from build123d import *

# Parameters (mm, degrees)
SKETCH_1_W                   = 64
SKETCH_1_H                   = 45
EXTRUDE_1_DEPTH              = 11.5
HOLE_WIZARD_M4_1_D           = 4.5
HOLE_WIZARD_M4_1_CBORE_D     = 8
HOLE_WIZARD_M4_1_CBORE_DEPTH = 4.4
FILLET_1_R                   = 3


with BuildPart() as part:
    # 草图1 → 凸台-拉伸1 (new, symmetric)
    with BuildSketch(Plane(origin=(0, 0, 0), x_dir=(1, 0, 0), z_dir=(0, 1, 0))):
        Rectangle(SKETCH_1_W, SKETCH_1_H)
    extrude(amount=EXTRUDE_1_DEPTH, both=True)

    # M4 六角凹头螺钉的柱形沉头孔1 (through all)
    with Locations(Plane(origin=(0, 11.5, 0), x_dir=(1, 0, 0), z_dir=(0, 1, 0))):
        with Locations((-23.5, 0), (23.5, 0)):
            CounterBoreHole(HOLE_WIZARD_M4_1_D / 2, HOLE_WIZARD_M4_1_CBORE_D / 2, HOLE_WIZARD_M4_1_CBORE_DEPTH)

    # 圆角1
    fillet_1_edges = [part.edges().sort_by_distance(p)[0] for p in [
        (32, 0, 22.5),
        (-32, 0, 22.5),
        (-32, 0, -22.5),
        (32, 0, -22.5),
    ]]
    fillet(fillet_1_edges, radius=FILLET_1_R)


solid = part.part
Could you check a few things on this model? Use its own coordinates, in mm. A direction names the side the tool comes from. Coordinates: 2 decimals unless noted, no trailing zeros. Loops run counter-clockwise (first coordinate to the right, second up) from the corner with the lowest first, then second, coordinate; pieces in that order, holes last.
1. For P1, Ø7, axis at x = 23.5, z = 0, coming from the +Y side, with a flat end and sliding along its axis, tell me the tip position at first contact or that it passes through.
2. Imagine slicing it at C-C (z = 0). Please give me the cut outline in (x, y), and give its area (3 significant figures).
3. Imagine slicing it at B-B (y = 8). Please give me the cut outline in (x, z).
4. For faces 4 (the face through (-22, 7.1, 2)), 5 (the face through (21.354, -2.33, -0.676)), which set-ups out of +Z, -Z, +X, -X, +Y, -Y let a thin tool reach every point of the face, with its end or its side?
5. I need wall thicknesses on L1, parallel to Z at x = 23.5, y = 8.8; L2, parallel to Z at x = 23.5, y = 2; L3, parallel to X at y = -6.25, z = 1. Which ranges of each line are inside material? Lowest first, please.
6. We'd pull the mould along Z, two halves only. Please class faces 1 (the face through (0, -11.5, 0)), 2 (the face through (0, 0, 22.5)), 3 (the face through (20.3, 9.3, 2.4)): released by +Z, released by -Z, zero draft, split by the parting line, or undercut.
7. Imagine slicing it at A-A (x = 23.5). Please give me the cut outline in (y, z).
Computed values:
1. P1: stops at y = 7.1
2. outline: (-32, -11.5) - (-25.75, -11.5) - (-25.75, 7.1) - (-27.5, 7.1) - (-27.5, 11.5) - (-32, 11.5) - close; (-21.25, -11.5) - (21.25, -11.5) - (21.25, 7.1) - (19.5, 7.1) - (19.5, 11.5) - (-19.5, 11.5) - (-19.5, 7.1) - (-21.25, 7.1) - close; (25.75, -11.5) - (32, -11.5) - (32, 11.5) - (27.5, 11.5) - (27.5, 7.1) - (25.75, 7.1) - close
2. area: 1,230 mm2
3. outline: (-32, -19.5) arc R3 ccw to (-29, -22.5) - (29, -22.5) arc R3 ccw to (32, -19.5) - (32, 19.5) arc R3 ccw to (29, 22.5) - (-29, 22.5) arc R3 ccw to (-32, 19.5) - close; hole circle Ø8 at (-23.5, 0); hole circle Ø8 at (23.5, 0)
4. face 4: +Y
4. face 5: +Y, -Y
5. L1: z = -22.5 to -4, 4 to 22.5
5. L2: z = -22.5 to -2.25, 2.25 to 22.5
5. L3: x = -32 to -25.52, -21.48 to 21.48, 25.52 to 32
6. face 1: zero draft
6. face 2: released by +Z
6. face 3: undercut
7. outline: (-11.5, -22.5) - (11.5, -22.5) - (11.5, -4) - (7.1, -4) - (7.1, -2.25) - (-11.5, -2.25) - close; (-11.5, 2.25) - (7.1, 2.25) - (7.1, 4) - (11.5, 4) - (11.5, 22.5) - (-11.5, 22.5) - close
